from build123d import *

# Parameters (mm, degrees)
SKETCH_1_W               = 150
SKETCH_1_H               = 180
EXTRUDE_1_DEPTH          = 18
CHAMFER_1_SIZE           = 10
HOLE_WIZARD_1_AT_2_COUNT = 2
HOLE_WIZARD_1_AT_2_PITCH = 33
HOLE_WIZARD_1_AT_3_COUNT = 2
HOLE_WIZARD_1_AT_3_PITCH = 87
HOLE_WIZARD_1_AT_4_COUNT = 2
HOLE_WIZARD_1_AT_4_PITCH = 120
HOLE_WIZARD_1_AT_5_COUNT = 2
HOLE_WIZARD_1_AT_5_PITCH = 124
HOLE_WIZARD_1_AT_6_COUNT = 2
HOLE_WIZARD_1_AT_6_PITCH = 128.316016148
HOLE_WIZARD_1_AT_7_COUNT = 2
HOLE_WIZARD_1_AT_7_PITCH = 151.476070717
HOLE_WIZARD_1_AT_8_COUNT = 2
HOLE_WIZARD_1_AT_8_PITCH = 172.557236881
SKETCH_6_R               = 3
CUT_EXTRUDE_1_DEPTH      = 119.528477591
HOLE_WIZARD_2_AT_2_COUNT = 2
HOLE_WIZARD_2_AT_2_PITCH = 40
HOLE_WIZARD_2_AT_3_COUNT = 2
HOLE_WIZARD_2_AT_3_PITCH = 92.135769384
HOLE_WIZARD_2_AT_4_COUNT = 2
HOLE_WIZARD_2_AT_4_PITCH = 83


with BuildPart() as part:
    # 草图1 → 凸台-拉伸1 (new body)
    with BuildSketch(Plane(origin=(0, 0, 0), x_dir=(1, 0, 0), z_dir=(0, 1, 0))):
        Rectangle(SKETCH_1_W, SKETCH_1_H)
    extrude(amount=EXTRUDE_1_DEPTH)

    # 倒角1
    chamfer_1_edges = [part.edges().sort_by_distance(p)[0] for p in [
        (75, 9, 90),
        (-75, 9, 90),
        (-75, 9, -90),
        (75, 9, -90),
    ]]
    chamfer(chamfer_1_edges, length=CHAMFER_1_SIZE)

    # 草图5 → 打孔尺寸(%根据)内六角圆柱头螺钉的类型1 (revolve, cut)
    with BuildSketch(Plane(origin=(60, 0, -46.999999026), x_dir=(0, 0, -1), z_dir=(1, 0, 0))):
        Polygon((0, 0), (0, 18), (3.3, 18), (3.3, 6.8), (5.5, 6.8), (5.5, 1.025), (6.525, 0), align=None)
    hole_wizard_1 = revolve(axis=Axis((60, -6.35, -46.999999026), (0, 1, 0)), mode=Mode.SUBTRACT)

    # 打孔尺寸(%根据)内六角圆柱头螺钉的类型1 at 2: 打孔尺寸(%根据)内六角圆柱头螺钉的类型1 ×2
    with Locations(*[(-i * HOLE_WIZARD_1_AT_2_PITCH, 0, 0) for i in range(1, HOLE_WIZARD_1_AT_2_COUNT)]):
        add(hole_wizard_1, mode=Mode.SUBTRACT)

    # 打孔尺寸(%根据)内六角圆柱头螺钉的类型1 at 3: 打孔尺寸(%根据)内六角圆柱头螺钉的类型1 ×2
    with Locations(*[(-i * HOLE_WIZARD_1_AT_3_PITCH, 0, 0) for i in range(1, HOLE_WIZARD_1_AT_3_COUNT)]):
        add(hole_wizard_1, mode=Mode.SUBTRACT)

    # 打孔尺寸(%根据)内六角圆柱头螺钉的类型1 at 4: 打孔尺寸(%根据)内六角圆柱头螺钉的类型1 ×2
    with Locations(*[(-i * HOLE_WIZARD_1_AT_4_PITCH, 0, 0) for i in range(1, HOLE_WIZARD_1_AT_4_COUNT)]):
        add(hole_wizard_1, mode=Mode.SUBTRACT)

    # 打孔尺寸(%根据)内六角圆柱头螺钉的类型1 at 5: 打孔尺寸(%根据)内六角圆柱头螺钉的类型1 ×2
    with Locations(*[(0, 0, i * HOLE_WIZARD_1_AT_5_PITCH) for i in range(1, HOLE_WIZARD_1_AT_5_COUNT)]):
        add(hole_wizard_1, mode=Mode.SUBTRACT)

    # 打孔尺寸(%根据)内六角圆柱头螺钉的类型1 at 6: 打孔尺寸(%根据)内六角圆柱头螺钉的类型1 ×2
    with Locations(*[Vector(-0.25717756045339407, 0, 0.9663641665538105) * (i * HOLE_WIZARD_1_AT_6_PITCH) for i in range(1, HOLE_WIZARD_1_AT_6_COUNT)]):
        add(hole_wizard_1, mode=Mode.SUBTRACT)

    # 打孔尺寸(%根据)内六角圆柱头螺钉的类型1 at 7: 打孔尺寸(%根据)内六角圆柱头螺钉的类型1 ×2
    with Locations(*[Vector(-0.5743481434915226, 0, 0.8186111470459227) * (i * HOLE_WIZARD_1_AT_7_PITCH) for i in range(1, HOLE_WIZARD_1_AT_7_COUNT)]):
        add(hole_wizard_1, mode=Mode.SUBTRACT)

    # 打孔尺寸(%根据)内六角圆柱头螺钉的类型1 at 8: 打孔尺寸(%根据)内六角圆柱头螺钉的类型1 ×2
    with Locations(*[Vector(-0.6954214275158859, 0, 0.7186021417667552) * (i * HOLE_WIZARD_1_AT_8_PITCH) for i in range(1, HOLE_WIZARD_1_AT_8_COUNT)]):
        add(hole_wizard_1, mode=Mode.SUBTRACT)

    # 草图6 → 切除-拉伸1 (cut, through all)
    with BuildSketch(Plane.XZ):
        with Locations(Location((0, -46.999999026, 0), (0, 0, 270))):
            Circle(SKETCH_6_R)
        with Locations(Location((0, 77.000000974, 0), (0, 0, 270))):
            Circle(SKETCH_6_R)
    extrude(amount=-CUT_EXTRUDE_1_DEPTH, mode=Mode.SUBTRACT)

    # 草图8 → 打孔尺寸(%根据)内六角圆柱头螺钉的类型2 (revolve, cut)
    with BuildSketch(Plane(origin=(-39, 18, -40), x_dir=(0, 0, 1), z_dir=(1, 0, 0))):
        Polygon((0, 0), (0, 18), (3.3, 18), (3.3, 6.8), (5.5, 6.8), (5.5, 0.9), (6.4, 0), align=None)
    hole_wizard_2 = revolve(axis=Axis((-39, 24.35, -40), (0, -1, 0)), mode=Mode.SUBTRACT)

    # 打孔尺寸(%根据)内六角圆柱头螺钉的类型2 at 2: 打孔尺寸(%根据)内六角圆柱头螺钉的类型2 ×2
    with Locations(*[(0, 0, -i * HOLE_WIZARD_2_AT_2_PITCH) for i in range(1, HOLE_WIZARD_2_AT_2_COUNT)]):
        add(hole_wizard_2, mode=Mode.SUBTRACT)

    # 打孔尺寸(%根据)内六角圆柱头螺钉的类型2 at 3: 打孔尺寸(%根据)内六角圆柱头螺钉的类型2 ×2
    with Locations(*[Vector(0.9008444880292467, 0, -0.4341419219418052) * (i * HOLE_WIZARD_2_AT_3_PITCH) for i in range(1, HOLE_WIZARD_2_AT_3_COUNT)]):
        add(hole_wizard_2, mode=Mode.SUBTRACT)

    # 打孔尺寸(%根据)内六角圆柱头螺钉的类型2 at 4: 打孔尺寸(%根据)内六角圆柱头螺钉的类型2 ×2
    with Locations(*[(i * HOLE_WIZARD_2_AT_4_PITCH, 0, 0) for i in range(1, HOLE_WIZARD_2_AT_4_COUNT)]):
        add(hole_wizard_2, mode=Mode.SUBTRACT)


solid = part.part
Here's how the part is built. I have some questions about the finished solid (model axes, mm). A direction names the side the tool comes from. Coordinates: 2 decimals unless noted, no trailing zeros. Order: outer loops, then holes, each group sorted by start corner. A loop starts at its lowest first (then second) coordinate and runs counter-clockwise, first axis right, second up.
Item 1: If we section it at B-B on y = 3: State how many separate pieces and enclosed holes the cut face has, plus the area to 3 significant figures.
Result sheet:
separate pieces: 1
enclosed holes: 14
area: 25,800 mm2
Item 2: If we mould it in two halves opening along X, with no side actions, what happens to faces 4 (the face through (70, 9, -85)), 5 (the face through (-39, 11.2, -84)), 6 (the face through (-1, 0, -1))? For each: +X half, -X half, draft (parallel to the pull), parting line (faces both ways), or undercut.
Result sheet:
face 4: +X half
face 5: undercut
face 6: draft
Item 3: For P1, Ø4, axis at x = -60, z = -47, coming from the -Y side; P2, Ø7.5, axis at x = -27, z = -47, coming from the -Y side; P3, Ø9, axis at x = 28.5, z = -46.5, coming from the -Y side; P4, Ø3.5, axis at x = -38.5, z = -38.5, coming from the +Y side, each with a flat end and sliding along its axis, tell me the tip position at first contact or that it passes through.
Result sheet:
P1: passes through
P2: stops at y = 6.8
P3: stops at y = 0.44
P4: stops at y = 11.2
Item 4: If we section it at A-A on x = 27: List the corners of the cut face in (y, z) for me (3 decimals).
Result sheet:
outline: (0, -90) - (18, -90) - (18, -50.3) - (6.8, -50.3) - (6.8, -52.5) - (1.025, -52.5) - (0, -53.525) - close; (0, -40.475) - (1.025, -41.5) - (6.8, -41.5) - (6.8, -43.7) - (18, -43.7) - (18, 73.7) - (6.8, 73.7) - (6.8, 71.5) - (1.025, 71.5) - (0, 70.475) - close; (0, 83.525) - (1.025, 82.5) - (6.8, 82.5) - (6.8, 80.3) - (18, 80.3) - (18, 90) - (0, 90) - close
Item 5: For faces 1 (the face through (-64.638, 3.872, 74.043)), 2 (the face through (-1, 18, -1)), 3 (the face through (-39.242, 14.191, -45.495)), which set-ups out of +Z, -Z, +X, -X, +Y, -Y let a thin tool reach every point of the face, with its end or its side?
Result sheet:
face 1: -Y
face 2: +Z, -Z, +X, -X, +Y
face 3: +Y
Item 6: I need wall thicknesses on line 1 (X direction, y = 2.75, z = -80); line 2 (Z direction, x = 44, y = 7.5); line 3 (X direction, y = 11, z = 77). Which ranges of each line are inside material? Lowest first, please.
Result sheet:
line 1: x = -75 to -42.3, -35.7 to 40.7, 47.3 to 75
line 2: z = -90 to -83.3, -76.7 to -43.3, -36.7 to 90
line 3: x = -75 to -63.3, -56.7 to -30.3, -23.7 to -3, 3 to 23.7, 30.3 to 56.7, 63.3 to 75
Item 7: If we section it at C-C on x = -39: List the corners of the cut face in (y, z) for me, plus the area to 3 significant figures.
Result sheet:
outline: (0, -90) - (18, -90) - (18, -86.4) - (17.1, -85.5) - (11.2, -85.5) - (11.2, -83.3) - (0, -83.3) - close; (0, -76.7) - (11.2, -76.7) - (11.2, -74.5) - (17.1, -74.5) - (18, -73.6) - (18, -46.4) - (17.1, -45.5) - (11.2, -45.5) - (11.2, -43.3) - (0, -43.3) - close; (0, -36.7) - (11.2, -36.7) - (11.2, -34.5) - (17.1, -34.5) - (18, -33.6) - (18, 90) - (0, 90) - close
area: 2,940 mm2
